Geometry: final body of the model. Coordinates: model frame, mm. A direction names the side the tool comes from. Give positions to 0.01 mm unless a question says otherwise; leave off trailing zeros. Loops run counter-clockwise (first coordinate to the right, second up) from the corner with the lowest first, then second, coordinate; pieces in that order, holes last. Notation, with made-up numbers: (-18, 19.5) - (-5, 19.5) arc R22 ccw to (-5, 46.5) - close; hole circle Ø6 at (85.5, 40). An arc over 180 degrees is marked (long way). Answer in a Markdown table with one row per item.
from build123d import *

# Parameters (mm, degrees)
BASE_BLOCK_PROFILE_W          = 100
BASE_BLOCK_PROFILE_H          = 19
BASE_BLOCK_100X19X48_DEPTH    = 24
END_NOTCHES_CUT_DEPTH         = 24
GUIDE_SLOT_63X3_DEPTH_1_DEPTH = 1
V_BLOCK_BODY_DEPTH            = 50
V_GROOVE_CUT_DEPTH            = 60
CROSS_HOLE_8_SKETCH_R         = 4
CROSS_HOLE_8_DEPTH            = 55
HOLE_10_SKETCH_R              = 5
HOLE_10_DEPTH                 = 60


with BuildPart() as part:
    # Base Block Profile → Base Block 100x19x48 (new, symmetric)
    with BuildSketch(Plane.XY):
        with Locations((50, 9.5)):
            Rectangle(BASE_BLOCK_PROFILE_W, BASE_BLOCK_PROFILE_H)
    extrude(amount=BASE_BLOCK_100X19X48_DEPTH, both=True)

    # End Notch Profile → End Notches Cut (cut, symmetric)
    with BuildSketch(Plane(origin=(0, 19, 0), x_dir=(1, 0, 0), z_dir=(0, 1, 0))):
        Polygon((100, -24), (100, -16.5), (89, -16.5), (89, -13.5), (84, -13.5), (84, -24), align=None)
        Polygon((100, -13.5), (100, 0), (84, 0), (84, -2), (89, -2), align=None)
        Polygon((100, 0), (100, 13.5), (89, 2), (84, 2), (84, 0), align=None)
        Polygon((100, 24), (84, 24), (84, 13.5), (89, 13.5), (89, 16.5), (100, 16.5), align=None)
    extrude(amount=END_NOTCHES_CUT_DEPTH, both=True, mode=Mode.SUBTRACT)

    # Guide Slot Sketch → Guide Slot 63x3 Depth 1 (cut)
    with BuildSketch(Plane(origin=(0, 19, 0), x_dir=(1, 0, 0), z_dir=(0, 1, 0))):
        with BuildLine():
            Line((60, -12.5), (60, 12.5))
            ThreePointArc((60, 12.5), (63, 15.5), (66, 12.5))
            Line((66, 12.5), (66, -12.5))
            ThreePointArc((66, -12.5), (63, -15.5), (60, -12.5))
        make_face()
    extrude(amount=-GUIDE_SLOT_63X3_DEPTH_1_DEPTH, mode=Mode.SUBTRACT)

    # V-Block Body Profile → V-Block Body (add)
    with BuildSketch(Plane.ZY):
        Polygon((-16.5, 19), (-16.5, 32), (-24, 32), (-24, 38), (-13.5, 38), (-13.5, 43), (-16.5, 43), (-16.5, 54), (-13.5, 54), (-1.5, 41), (-1.5, 38), (1.5, 38), (1.5, 41), (13.5, 54), (16.5, 54), (16.5, 43), (13.5, 43), (13.5, 38), (24, 38), (24, 32), (16.5, 32), (16.5, 19), align=None)
    extrude(amount=-V_BLOCK_BODY_DEPTH)

    # V-Groove Sketch → V-Groove Cut (cut)
    with BuildSketch(Plane.XY.offset(24)):
        Polygon((50, 19), (52.80194455, 14.895599546), (55.491811317, 19), align=None)
    extrude(amount=-V_GROOVE_CUT_DEPTH, mode=Mode.SUBTRACT)

    # Cross Hole Ø8 Sketch → Cross Hole Ø8 (cut, symmetric)
    with BuildSketch(Plane(origin=(0, 38, 0), x_dir=(1, 0, 0), z_dir=(0, 1, 0))):
        with Locations(Location((25, 0, 0), (0, 0, 270))):
            Circle(CROSS_HOLE_8_SKETCH_R)
    extrude(amount=CROSS_HOLE_8_DEPTH, both=True, mode=Mode.SUBTRACT)

    # Hole Ø10 Sketch → Hole Ø10 (cut)
    with BuildSketch(Plane.XY.offset(24)):
        with Locations(Location((25, 25, 0), (0, 0, 90))):
            Circle(HOLE_10_SKETCH_R)
    extrude(amount=-HOLE_10_DEPTH, mode=Mode.SUBTRACT)


solid = part.part
Q1. Cut plane B-B (x = 25). Give the number of separate pieces and of enclosed holes in the cut face, and give its area (3 significant figures).
Check values:
| item | result |
|---|---|
| separate pieces | 4 |
| enclosed holes | 0 |
| area | 1,350 mm² |
Q2. Cut plane D-D (z = -11). Output: boundary loops of the cut face in (x, y), and give its area (3 significant figures).
Check values:
| item | result |
|---|---|
| outline | (0, 0) - (97.61, 0) - (97.61, 19) - (66, 19) - (66, 18) - (60, 18) - (60, 19) - (55.49, 19) - (52.8, 14.9) - (50, 19) - (50, 51.29) - (0, 51.29) - close; hole circle Ø10 at (25, 25) |
| area | 3,370 mm² |
Q3. Material intervals for line 1 along X through (y, z) = (33.5, 0); line 2 along Z through (x, y) = (86.5, 4.5); line 3 along Z through (x, y) = (25, 40), sorted ascending.
Check values:
| item | result |
|---|---|
| line 1 | 0 to 21, 29 to 50 |
| line 2 | -13.5 to -2, 2 to 13.5 |
| line 3 | -13.5 to -4, 4 to 13.5 |
Q4. Reachability of faces 4 (the flat face through (25, 38, -19)), 5 (the flat face through (25, 48, -16.5)), 6 (the flat face through (24.65, 47.409, 7.416)), 7 (the flat face through (89, 10, -15)), 8 (the flat face through (94.577, 9.367, -7.83)) from +Z, -Z, +X, -X, +Y, -Y: full face, straight path, thin tool, end or side. Return the list, or none.
Check values:
| item | result |
|---|---|
| face 4 | -Z, +X, -X |
| face 5 | -Z, +X, -X, +Y |
| face 6 | +X, -X, +Y |
| face 7 | -Z, +Y, -Y |
| face 8 | +X, +Y, -Y |
Q5. First-contact query: pin 1 (3.5 mm diameter, centred on x = 42.5, z = 0, fed in from +Y); pin 2 (2 mm diameter, centred on x = 10, z = -9.5, fed in from +Y); pin 3 (1.1 mm diameter, centred on y = 18.5, z = 5.5, fed in from +X). Flat tips, straight axial feed; report the tip coordinate or a pass-through.
Check values:
| item | result |
|---|---|
| pin 1 | y = 41.27 |
| pin 2 | y = 50.75 |
| pin 3 | x = 92.87 |
Q6. Cut plane C-C (y = 13.5). Output: boundary loops of the cut face in (x, z).
Check values:
| item | result |
|---|---|
| outline | (0, -24) - (84, -24) - (84, -13.5) - (89, -13.5) - (89, -16.5) - (100, -16.5) - (100, -13.5) - (89, -2) - (84, -2) - (84, 2) - (89, 2) - (100, 13.5) - (100, 16.5) - (89, 16.5) - (89, 13.5) - (84, 13.5) - (84, 24) - (0, 24) - close; hole circle Ø8 at (25, 0) |
Q7. Draft query along X for faces 1 (the flat face through (50, 33, 0)), 2 (the flat face through (49, 0, 0)), 3 (the flat face through (51.38, 16.98, 0.34)). Return one class per face: pulls with the +X half, pulls with the -X half, needs draft (parallel to the pull), parting line crosses it, or undercut.
Check values:
| item | result |
|---|---|
| face 1 | pulls with the +X half |
| face 2 | needs draft |
| face 3 | undercut |
Q8. Cut plane A-A (y = 25). Output: boundary loops of the cut face in (x, z), and give its area (3 significant figures).
Check values:
| item | result |
|---|---|
| outline | (0, -16.5) - (20, -16.5) - (20, 16.5) - (0, 16.5) - close; (30, -16.5) - (50, -16.5) - (50, 16.5) - (30, 16.5) - close |
| area | 1,320 mm² |
